Check sheet for the modelled part. Datum: model origin and axes. Units: mm. Face numbers are marked on the shaded views. A direction names the side the tool comes from. Give positions to 0.01 mm unless a question says otherwise; leave off trailing zeros. Write each loop counter-clockwise with the first axis right and the second up, starting at its lowest first coordinate (ties: lowest second). Pieces come first, ordered by that corner, then holes. Notation, with made-up numbers: M -18,-30.75 L -3,-30.75 A10 ccw -3,-18.75 Z; hole C -10.75,52 d9. An arc over 180 degrees is marked long. One line per item, written item: value. Start each with the question number.
from build123d import *


with BuildPart() as part:
    # Sketch1 → Revolve1 (revolve)
    with BuildSketch(Plane.XY):
        Polygon((0, 303), (-6, 303), (-6, 288), (-7, 288), (-7, 243), (-7.5, 243), (-7.5, 233), (-9, 233), (-9, 195), (-11, 195), (-11, 170), (-14, 170), (-14, 165), (-9, 165), (-9, 72), (-7.5, 72), (-7.5, 60), (-7, 60), (-7, 15), (-6, 15), (-6, 0), (0, 0), align=None)
    revolve(axis=Axis((0, 303, 0), (0, -1, 0)))


solid = part.part
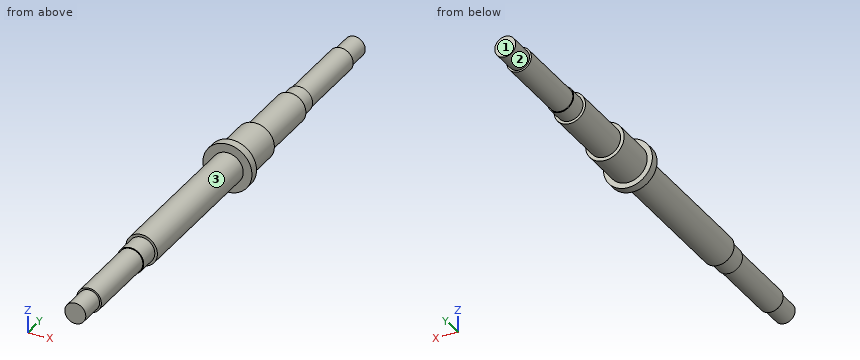
1) Material ranges on L1, parallel to Y at x = 5, z = 9.5; L2, parallel to Y at x = 0.75, z = 6.5; L3, parallel to X at y = 123, z = 0.5, recorded low to high. Write a range as from..to.
2) Tool access check on the marked faces 1, 2 and 3. Record the directions out of +Z, -Z, +X, -X, +Y, -Y that give a thin tool (end or side, any length) a straight path to the whole face; none if there is none.
3) Gauge pin test, flat ends, axial feed: pin 1 (12 mm diameter, centred on x = -8.5, y = 147.5, fed in from -Z); pin 2 (8 mm diameter, centred on x = -6.5, y = 249.5, fed in from +Z); pin 3 (1 mm diameter, centred on y = 169.5, z = -10, fed in from +X). Record the tip position at first contact, or that the pin passes through.
4) Cross-section at B-B (y = 199). Record the boundary of the cut face in (x, z), plus the area to 3 significant figures.
5) Cross-section at A-A (y = 19). Record the boundary of the cut face in (x, z).
Data:
1. L1: y = 165..195
1. L2: y = 15..288
1. L3: x = -8.99..8.99
2. face 1: +Z, -Z, +X, -X, +Y
2. face 2: +Y
2. face 3: -Y
3. pin 1: stops at z = -8.65
3. pin 2: stops at z = 6.54
3. pin 3: stops at x = 10.28
4. outline: C 0,0 d18
4. area: 254 mm2
5. outline: C 0,0 d14
